```python
from build123d import *

# Parameters (mm, degrees)
BOSS_EXTRUDE1_DEPTH = 8
SKETCH2_R           = 52.5
BOSS_EXTRUDE2_DEPTH = 45
SKETCH3_R           = 52.5
SKETCH3_R_2         = 50.75
CUT_EXTRUDE1_DEPTH  = 6
SKETCH4_R           = 32.5
CUT_EXTRUDE2_DEPTH  = 98.75607398
CHAMFER1_SIZE       = 2
CHAMFER2_SIZE       = 1.5
SKETCH5_OUTSIDE_W   = 889.986
SKETCH5_OUTSIDE_H   = 904.986
SKETCH5_OUTSIDE_R   = 55
CUT_EXTRUDE3_DEPTH  = 98.75607398
CUT_EXTRUDE3_DRAFT  = -75


with BuildPart() as part:
    # Sketch1 → Boss-Extrude1 (new body)
    with BuildSketch(Plane.XY):
        with BuildLine():
            ThreePointArc((-2.5, -64.951905284), (0, -65), (2.5, -64.951905284))
            Line((2.5, -64.951905284), (55, -34.641016151))
            ThreePointArc((55, -34.641016151), (56.291651246, -32.5), (57.5, -30.310889132))
            Line((57.5, -30.310889132), (57.5, 30.310889132))
            ThreePointArc((57.5, 30.310889132), (56.291651246, 32.5), (55, 34.641016151))
            Line((55, 34.641016151), (2.5, 64.951905284))
            ThreePointArc((2.5, 64.951905284), (0, 65), (-2.5, 64.951905284))
            Line((-2.5, 64.951905284), (-55, 34.641016151))
            ThreePointArc((-55, 34.641016151), (-56.291651246, 32.5), (-57.5, 30.310889132))
            Line((-57.5, 30.310889132), (-57.5, -30.310889132))
            ThreePointArc((-57.5, -30.310889132), (-56.291651246, -32.5), (-55, -34.641016151))
            Line((-55, -34.641016151), (-2.5, -64.951905284))
        make_face()
    extrude(amount=BOSS_EXTRUDE1_DEPTH)

    # Sketch2 → Boss-Extrude2 (add)
    with BuildSketch(Plane(origin=(0, 0, 0), x_dir=(-1, 0, 0), z_dir=(0, 0, -1))):
        Circle(SKETCH2_R)
    extrude(amount=-BOSS_EXTRUDE2_DEPTH)

    # Sketch3 → Cut-Extrude1 (cut)
    with BuildSketch(Plane.XY.offset(8)):
        with Locations(Location((0, 0, 0), (0, 0, 180))):
            Circle(SKETCH3_R)
        Circle(SKETCH3_R_2, mode=Mode.SUBTRACT)
    extrude(amount=CUT_EXTRUDE1_DEPTH, mode=Mode.SUBTRACT)

    # Sketch4 → Cut-Extrude2 (cut, through all)
    with BuildSketch(Plane.XY.offset(45)):
        Circle(SKETCH4_R)
    extrude(amount=-CUT_EXTRUDE2_DEPTH, mode=Mode.SUBTRACT)

    # Chamfer1
    chamfer1_edges = [part.edges().sort_by_distance(p)[0] for p in [
        (-32.5, 0, 0),
        (-32.5, 0, 45),
    ]]
    chamfer(chamfer1_edges, length=CHAMFER1_SIZE)

    # Chamfer2
    chamfer2_edges = [part.edges().sort_by_distance(p)[0] for p in [
        (52.5, 0, 45),
    ]]
    chamfer(chamfer2_edges, length=CHAMFER2_SIZE)


with BuildPart() as cut_extrude3_tool:
    # Sketch5 outside → Cut-Extrude3 (with draft: the straight prism first)
    with BuildSketch(Plane(origin=(0, 0, 0), x_dir=(-1, 0, 0), z_dir=(0, 0, -1))):
        Rectangle(SKETCH5_OUTSIDE_W, SKETCH5_OUTSIDE_H)
        Circle(SKETCH5_OUTSIDE_R, mode=Mode.SUBTRACT)
    extrude(amount=-CUT_EXTRUDE3_DEPTH)
    # Cut-Extrude3: the draft: its side faces are tilted about the plane it starts from
    cut_extrude3_sides = [cut_extrude3_tool.faces().sort_by_distance(p)[0] for p in [
        (0, -452.493, 49.37803699),
        (-444.993, 0, 49.37803699),
        (0, 452.493, 49.37803699),
        (444.993, 0, 49.37803699),
        (55, 0, 49.37803699),
    ]]
    draft(cut_extrude3_sides, Plane(origin=(0, 0, 0), x_dir=(-1, 0, 0), z_dir=(0, 0, -1)), CUT_EXTRUDE3_DRAFT)


with BuildPart() as part_1:
    add(part.part)

    # Cut-Extrude3: cut by cut_extrude3_tool
    add(cut_extrude3_tool.part, mode=Mode.SUBTRACT)


solid = part_1.part
```
Could you check a few things on this model? Use its own coordinates, in mm. A direction names the side the tool comes from. Round coordinates to 2 decimals unless told otherwise and drop trailing zeros. Loops run counter-clockwise (first coordinate to the right, second up) from the corner with the lowest first, then second, coordinate; pieces in that order, holes last. Notation, with made-up numbers: M 25,88 L 68,88 A26 cw 68,103 Z; hole C 50,-7.5 d2. An arc over 180 degrees is marked long. Put each result on its own line as item: value.
Q1. I need wall thicknesses on probe 1 along Y at (x, z) = (0, 12); probe 2 along Y at (x, z) = (0, 23); probe 3 along Z at (x, y) = (39, 38). Which ranges of each line are inside material? Lowest first, please.
Check result:
probe 1: -50.75 to -32.5, 32.5 to 50.75
probe 2: -52.5 to -32.5, 32.5 to 52.5
probe 3: 0 to 8
Q2. Thinking about a two-plate mould opening in X: for faces 3 (the face through (-50.076, 15.77, 28.544)), 4 (the face through (31, 9.76, 22.79)), 5 (the face through (-56, 33, 5)), which applies, released by +X, released by -X, zero draft, split by the parting line, or undercut?
Check result:
face 3: split by the parting line
face 4: undercut
face 5: released by -X
Q3. On a 3-axis mill with a long thin cutter (end or side, diameter ignored), from which of +Z, -Z, +X, -X, +Y, -Y can I reach the whole of each face in a straight line? I mean faces 1 (the face through (-56.31, -32.47, 5.3)), 2 (the face through (48.406, 15.244, 10.958)). Say none if no direction works.
Check result:
face 1: +Z, -Z, -X, -Y
face 2: none
Q4. Imagine slicing it at B-B (y = 0). Write out the boundary of the cut face in (x, z).
Check result:
outline: M -57.5,0.67 L -55,0 L -34.5,0 L -32.5,2 L -32.5,43 L -34.5,45 L -51,45 L -52.5,43.5 L -52.5,14 L -50.75,14 L -50.75,8 L -57.5,8 Z; M 32.5,2 L 34.5,0 L 55,0 L 57.5,0.67 L 57.5,8 L 50.75,8 L 50.75,14 L 52.5,14 L 52.5,43.5 L 51,45 L 34.5,45 L 32.5,43 Z
Q5. Imagine slicing it at A-A (x = 0). Write out the boundary of the cut face in (y, z), then the cut area to 3 significant figures.
Check result:
outline: M -65,2.68 L -55,0 L -34.5,0 L -32.5,2 L -32.5,43 L -34.5,45 L -51,45 L -52.5,43.5 L -52.5,14 L -50.75,14 L -50.75,8 L -65,8 Z; M 32.5,2 L 34.5,0 L 55,0 L 65,2.68 L 65,8 L 50.75,8 L 50.75,14 L 52.5,14 L 52.5,43.5 L 51,45 L 34.5,45 L 32.5,43 Z
area: 1,940 mm2
Q6. Imagine slicing it at C-C (z = 12.5). Write out the boundary of the cut face in (x, y).
Check result:
outline: C 0,0 d101.5; hole C 0,0 d65
Q7. For pin 1 (2 mm diameter, centred on x = -30.5, y = -3, fed in from +Z); pin 2 (12 mm diameter, centred on x = -41.5, y = 42.5, fed in from +Z); pin 3 (2 mm diameter, centred on y = -27.5, z = 9.5, fed in from +X); pin 4 (1 mm diameter, centred on x = 33.5, z = 25.5, fed in from -Y), each with a flat end and sliding along its axis, tell me the tip position at first contact or that it passes through.
Check result:
pin 1: through
pin 2: z = 8
pin 3: x = 43.28
pin 4: y = -40.83
